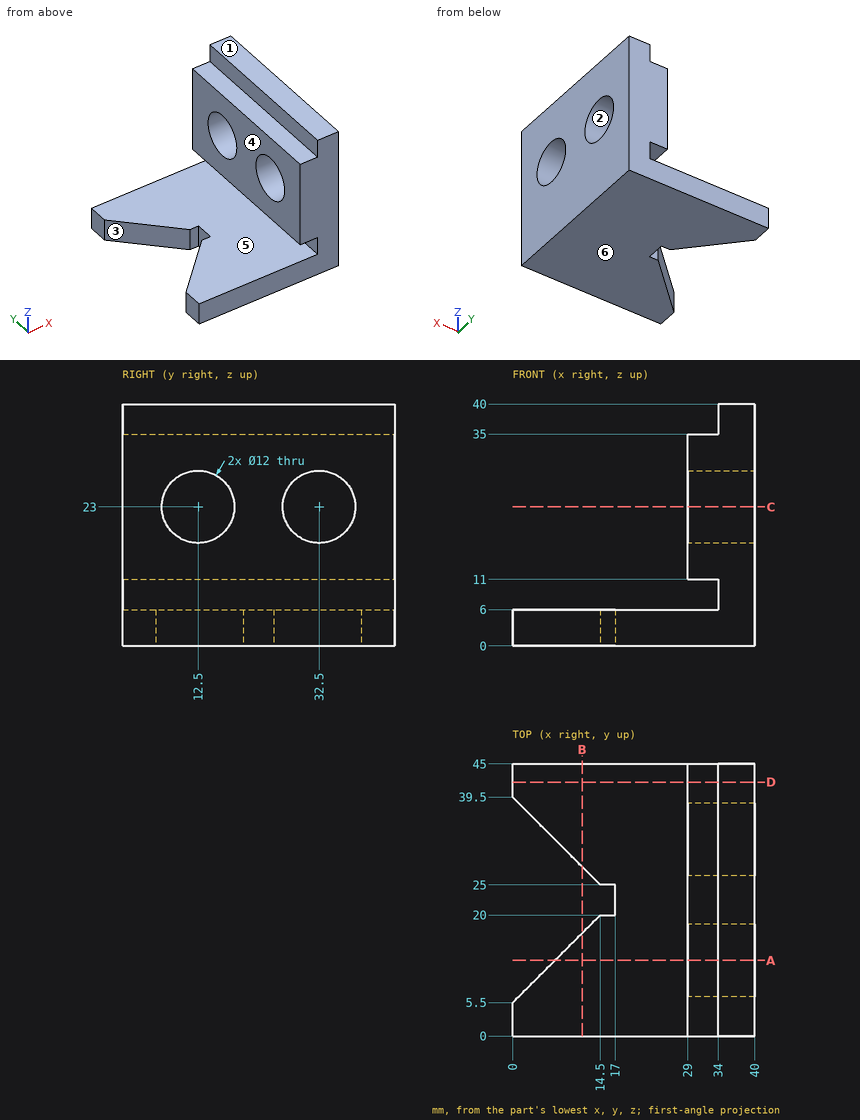
Print and shaded views of the part. All mm, measured from the part's lowest x, y and z. A direction names the side the tool comes from. Round coordinates to 2 decimals unless told otherwise and drop trailing zeros. Write each loop counter-clockwise with the first axis right and the second up, starting at its lowest first coordinate (ties: lowest second). Pieces come first, ordered by that corner, then holes. Notation, with made-up numbers: (34.25, -27) - (84.25, -27) arc R17 cw to (84.25, 5) - close; hole circle Ø1 at (8.25, -38). An arc over 180 degrees is marked (long way). One line per question, with ' | ' between items.
1. Drill centre lines: line 1 along Y through (x, z) = (32.5, 23); line 2 along Z through (x, y) = (30.5, 2.5); line 3 along X through (y, z) = (13, 30). Where is each one in solid material? Low to high. Write a range as from..to.
Results are:
line 1: 0..6.5, 18.5..26.5, 38.5..45 | line 2: 0..6, 11..35 | line 3: 29..40
2. Band-saw the part on C-C, the plane z = 23. Write the cut outline in (x, y), and give its area (3 significant figures).
Results are:
outline: (29, 0) - (40, 0) - (40, 6.5) - (29, 6.5) - close; (29, 18.5) - (40, 18.5) - (40, 26.5) - (29, 26.5) - close; (29, 38.5) - (40, 38.5) - (40, 45) - (29, 45) - close | area: 231 mm^2
3. Band-saw the part on D-D, the plane y = 42. Write the cut outline in (x, z), and give its area (3 significant figures).
Results are:
outline: (0, 0) - (40, 0) - (40, 40) - (34, 40) - (34, 35) - (29, 35) - (29, 11) - (34, 11) - (34, 6) - (0, 6) - close | area: 564 mm^2
4. Drop flat-ended pins along their axis: pin 1 Ø2.5 at (y, z) = (23, 3.5) entering from -X; pin 2 Ø1.5 at (x, y) = (13.5, 23.5) entering from +Z; pin 3 Ø5 at (x, y) = (31, 40.5) entering from +Z; pin 4 Ø5.5 at (y, z) = (15, 37) entering from -X. Give the stop position or say it passes through.
Results are:
pin 1: x = 17 | pin 2: through | pin 3: z = 35 | pin 4: x = 29
5. Tool access for the marked faces 4, 5 and 6: list every direction of +Z, -Z, +X, -X, +Y, -Y with a clear straight run to the whole face (end or side of a thin tool).
Results are:
face 4: +Z, -X, +Y, -Y | face 5: -X, +Y, -Y | face 6: -Z, +X, -X, +Y, -Y
6. Band-saw the part on A-A, the plane y = 12.5. Write the cut outline in (x, z).
Results are:
outline: (7, 0) - (40, 0) - (40, 17) - (29, 17) - (29, 11) - (34, 11) - (34, 6) - (7, 6) - close; (29, 29) - (40, 29) - (40, 40) - (34, 40) - (34, 35) - (29, 35) - close
7. Band-saw the part on B-B, the plane x = 11.5. Write the cut outline in (y, z).
Results are:
outline: (0, 0) - (17, 0) - (17, 6) - (0, 6) - close; (28, 0) - (45, 0) - (45, 6) - (28, 6) - close
8. Mould opens along Z. For the marked faces 1, 2 and 3 say: released by +Z, released by -Z, zero draft, split by the parting line, or undercut.
Results are:
face 1: released by +Z | face 2: undercut | face 3: zero draft
